Here's how the part is built. I have some questions about the finished solid (model axes, mm). A direction names the side the tool comes from. Round coordinates to 2 decimals unless told otherwise and drop trailing zeros. Write each loop counter-clockwise with the first axis right and the second up, starting at its lowest first coordinate (ties: lowest second). Pieces come first, ordered by that corner, then holes. Notation, with made-up numbers: (-29, 18) - (28, 18) arc R20 cw to (28, 38) - close; hole circle Ø11 at (5, 58). An arc over 180 degrees is marked (long way). One line per item, written item: value. Start each with the question number.
Item 1: Imagine slicing it at C-C, the plane y = -29.5. Please give me the cut outline in (x, z).
Item 2: Imagine slicing it at B-B, the plane x = -8.5. Please give me the cut outline in (y, z).
Item 3: For P1, Ø8, axis at x = -31, y = -18.5, coming from the +Z side; P2, Ø10, axis at x = -14.5, z = -2.5, coming from the -Y side; P3, Ø16, axis at x = -6, z = 19, coming from the +Y side; P4, Ø3, axis at y = -41.5, z = -82, coming from the +X side, each with a flat end and sliding along its axis, tell me the tip position at first contact or that it passes through.
Item 4: For faces 3 (the face through (-59.99, -40.88, -1.4)), 4 (the face through (-23, -85, -100)), 5 (the face through (-23, 3, -100)), which set-ups out of +Z, -Z, +X, -X, +Y, -Y let a thin tool reach every point of the face, with its end or its side?
Item 5: Thinking about a two-plate mould opening in Z: for faces 1 (the face through (0, -39, -2)), 2 (the face through (-23, -85, 100)), which applies, released by +Z, released by -Z, zero draft, split by the parting line, or undercut?
Item 6: If I drill on line 1 (Z direction, x = -26, y = 7.5); line 2 (X direction, y = -38, z = 41); line 3 (Y direction, x = -15, z = 18), over which ranges is the centre line in solid material (lowest first)?
Item 7: Imagine slicing it at D-D, the plane z = -70.5. Please give me the cut outline in (x, y).
Item 8: Imagine slicing it at A-A, the plane y = 8.5. Please give me the cut outline in (x, z), then the cut area to 3 significant figures.
```python
from build123d import *

# Parameters (mm, degrees)
EXTRUDE_1_DEPTH = 100
REVOLVE_1_ANGLE = 90


with BuildPart() as part:
    # 草图1 → 凸台-拉伸1 (new body)
    with BuildSketch(Plane.XY):
        with BuildLine():
            Line((0, 0), (0, -80))
            Line((0, -80), (-20, -80))
            ThreePointArc((-20, -80), (-60, -40), (-20, 0))
            Line((-20, 0), (0, 0))
        make_face()
    extrude_1 = extrude(amount=-EXTRUDE_1_DEPTH)

    # 草图2 → 旋转1 (revolve)
    with BuildSketch(Plane(origin=(0, 0, 0), x_dir=(0, 0, -1), z_dir=(1, 0, 0))):
        with BuildLine():
            Line((100, 20), (100, -100))
            ThreePointArc((100, -100), (160, -40), (100, 20))
        make_face()
    revolve_1 = revolve(axis=Axis((0, 20, -100), (0, 1, 0)), revolution_arc=REVOLVE_1_ANGLE)

    # 镜向1: 凸台-拉伸1, 旋转1 across plane
    add(extrude_1.mirror(Plane(origin=(-20, -40, 0), x_dir=(1, 0, 0), z_dir=(0, 0, -1))))
    add(revolve_1.mirror(Plane(origin=(-20, -40, 0), x_dir=(1, 0, 0), z_dir=(0, 0, -1))))


solid = part.part
```
Values follow:
1. outline: (-59.07, -100) arc R59.07 ccw to (0, -159.07) - (0, 159.07) arc R59.07 ccw to (-59.07, 100) - (-58.6, 100) - (-58.6, -100) - close
2. outline: (-99.39, -100) arc R59.39 ccw to (19.39, -100) - (0, -100) - (0, 100) - (19.39, 100) arc R59.39 ccw to (-99.39, 100) - (-80, 100) - (-80, -100) - close
3. P1: stops at z = 149.62
3. P2: stops at y = -80
3. P3: stops at y = 0
3. P4: stops at x = 0
4. face 3: -X
4. face 4: -X, -Y
4. face 5: -X, +Y
5. face 1: zero draft
5. face 2: undercut
6. line 1: z = -125.84 to -100, 100 to 125.84
6. line 2: x = -59.95 to 0
6. line 3: y = -80 to 0
7. outline: (-20, -80) - (0, -80) - (0, 0) - (-20, 0) arc R40 ccw to start
8. outline: (-35.32, -100) arc R35.32 ccw to (0, -135.32) - (0, -100) - close; (-35.32, 100) - (0, 100) - (0, 135.32) arc R35.32 ccw to start
8. area: 1,960 mm^2
